For this review, take the finished solid that the model builds, in its own axes (mm). Face numbers are marked on the shaded views. A direction names the side the tool comes from. Round coordinates to 2 decimals unless told otherwise and drop trailing zeros. Loops run counter-clockwise (first coordinate to the right, second up) from the corner with the lowest first, then second, coordinate; pieces in that order, holes last. Notation, with made-up numbers: M -2.75,-0.75 L 45.25,-0.75 A18 cw 45.25,24.25 Z; hole C 30.5,-21 d2. An arc over 180 degrees is marked long. One line per question, with ' | ' between items. Start each with the question number.
1) We need section C-C (x = 0). Give the boundary of the cut face in (y, z).
2) Mouldability with a two-part tool opening along Y and no side actions: class the marked faces 3, 4 and 5 as pulls with the +Y half, pulls with the -Y half, needs draft (parallel to the pull), parting line crosses it, or undercut.
3) For probe 1 along Y at (x, z) = (0.5, -12); probe 2 along Z at (x, y) = (-4.75, 14); probe 3 along Y at (x, z) = (4, -11), list the stretches that pass through material, from the lowest coordinate up. Write a range as from..to.
4) For the marked faces 1 and 2, list the 3-axis set-ups (+Z, -Z, +X, -X, +Y, -Y) from which the entire face can be reached by the end or side of a thin tool; tool diameter is ignored.
5) For pin 1 Ø6 at (x, y) = (4, 4.5) entering from +Z; pin 2 Ø2.5 at (x, z) = (-1, -0.5) entering from -Y; pin 3 Ø5 at (y, z) = (5, 6.5) entering from +X, all flat-tipped, find the tip position at first contact; note any pin that passes through.
6) We need section A-A (y = 13). Give the boundary of the cut face in (x, z).
7) We need section B-B (z = -12). Give the boundary of the cut face in (x, y).
8) We need section D-D (y = 8.75). Give the boundary of the cut face in (x, z).
```python
from build123d import *

# Parameters (mm, degrees)
EXTRUDE_1_DEPTH     = 23
SKETCH_2_R          = 2.5
CUT_EXTRUDE_1_DEPTH = 12
SKETCH_3_R          = 2.5
CUT_EXTRUDE_2_DEPTH = 62
CUT_EXTRUDE_3_DEPTH = 26


with BuildPart() as part:
    # 草图1 → 凸台-拉伸1 (new body)
    with BuildSketch(Plane(origin=(0, 0, 0), x_dir=(1, 0, 0), z_dir=(0, 1, 0))):
        with BuildLine():
            Line((-10, 0), (-10, 20))
            Line((-10, 20), (10, 20))
            Line((10, 20), (10, 0))
            ThreePointArc((10, 0), (0, -10), (-10, 0))
        make_face()
    extrude(amount=EXTRUDE_1_DEPTH)

    # 草图2 → 切除-拉伸1 (cut)
    with BuildSketch(Plane.XZ):
        with Locations(Location((0, 0, 0), (0, 0, 270))):
            Circle(SKETCH_2_R)
    extrude(amount=-CUT_EXTRUDE_1_DEPTH, mode=Mode.SUBTRACT)

    # 草图3 → 切除-拉伸2 (cut)
    with BuildSketch(Plane(origin=(10, 0, 0), x_dir=(0, 0, -1), z_dir=(1, 0, 0))):
        with Locations((12, 13)):
            Circle(SKETCH_3_R)
    extrude(amount=-CUT_EXTRUDE_2_DEPTH, mode=Mode.SUBTRACT)

    # 草图4 → 切除-拉伸3 (cut)
    with BuildSketch(Plane(origin=(10, 0, 0), x_dir=(0, 0, -1), z_dir=(1, 0, 0))):
        Polygon((0, 23), (-10, 23), (-10, 16.096925585), (4.676984075, 23), align=None)
    extrude(amount=-CUT_EXTRUDE_3_DEPTH, mode=Mode.SUBTRACT)


solid = part.part
```
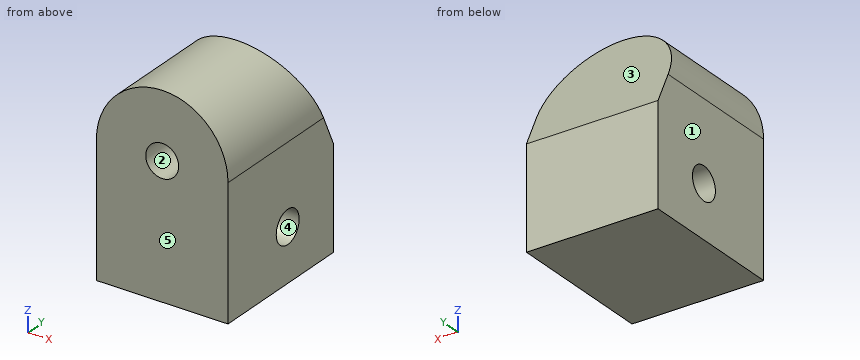
Answers below:
1) outline: M 0,-20 L 23,-20 L 23,-4.68 L 16.1,10 L 0,10 L 0,2.5 L 12,2.5 L 12,-2.5 L 0,-2.5 Z; hole C 13,-12 d5
2) face 3: pulls with the +Y half | face 4: undercut | face 5: pulls with the -Y half
3) probe 1: 0..10.5, 15.5..23 | probe 2: -20..-14.29, -9.71..8.8 | probe 3: 0..10.71, 15.29..23
4) face 1: +Z, -Z, -X, +Y, -Y | face 2: -Y
5) pin 1: z = 9.95 | pin 2: y = 12 | pin 3: x = 9.17
6) outline: M -10,-20 L 10,-20 L 10,-14.5 L -10,-14.5 Z; M -10,-9.5 L 10,-9.5 L 10,0 A10 ccw -10,0 Z
7) outline: M -10,0 L 10,0 L 10,10.5 L -10,10.5 Z; M -10,15.5 L 10,15.5 L 10,23 L -10,23 Z
8) outline: M -10,-20 L 10,-20 L 10,0 A10 ccw -10,0 Z; hole C 0,0 d5
